Here's how the part is built. I have some questions about the finished solid (model axes, mm). A direction names the side the tool comes from. Round coordinates to 2 decimals unless told otherwise and drop trailing zeros. Loops run counter-clockwise (first coordinate to the right, second up) from the corner with the lowest first, then second, coordinate; pieces in that order, holes last. Notation, with made-up numbers: (71, 69) - (116, 69) arc R27 cw to (116, 89) - close; hole circle Ø1 at (88.25, 80.25). An arc over 180 degrees is marked (long way). Return JSON: item names as keys, results as strings. Group by question number.
```python
from build123d import *

# Parameters (mm, degrees)
BASE_PLATE_DEPTH               = 56
HUB_BOSS_PROFILE_R             = 25
HUB_BOSS_PROFILE_R_2           = 12.5
HUB_BOSS_27_DEPTH              = 33
HUB_BORE_PROFILE_R             = 12.5
HUB_BORE_DEPTH                 = 186.162091153
FLANGE_START                   = 5
FLANGE_PLATE_PROFILE_R         = 6
FLANGE_PLATE_DEPTH             = 5
BASE_MOUNTING_HOLE_1_PROFILE_R = 8
BASE_MOUNTING_HOLE_1_DEPTH     = 209.137574695
BASE_MOUNTING_HOLE_2_PROFILE_R = 8
BASE_MOUNTING_HOLE_2_DEPTH     = 209.137574695
HUB_TO_BASE_FILLET_R5_R        = 5
FLANGE_FILLET_R5_R             = 5


with BuildPart() as part:
    # Base Plate Profile → Base Plate (new body)
    with BuildSketch(Plane.XY):
        Polygon((0, 0), (75, 0), (165, 0), (165, 16), (0, 16), align=None)
    extrude(amount=BASE_PLATE_DEPTH)

    # Hub Boss Profile → Hub Boss Ø27 (add, symmetric)
    with BuildSketch(Plane.XY.offset(25)):
        with Locations((82.5, 27)):
            Circle(HUB_BOSS_PROFILE_R)
        with Locations((82.5, 27)):
            Circle(HUB_BOSS_PROFILE_R_2, mode=Mode.SUBTRACT)
    extrude(amount=HUB_BOSS_27_DEPTH, both=True)

    # Hub Bore Profile → Hub Bore (cut, through all)
    with BuildSketch(Plane.XY.offset(58)):
        with Locations((82.5, 27)):
            Circle(HUB_BORE_PROFILE_R)
    extrude(amount=-HUB_BORE_DEPTH, mode=Mode.SUBTRACT)

    # Flange Plate Profile → Flange Plate (add)
    # profile 1 of 2: a face of its own
    with BuildSketch(Plane.XY.offset(51).offset(FLANGE_START)):
        with BuildLine():
            ThreePointArc((82.5, 87), (71.893398282, 91.393398282), (67.5, 102))
            Line((67.5, 102), (67.5, 47))
            ThreePointArc((67.5, 47), (82.5, 52), (97.5, 47))
            Line((97.5, 47), (97.5, 85.094750193))
            ThreePointArc((97.5, 85.094750193), (90.060257549, 86.521781776), (82.5, 87))
        make_face()
    # profile 2 of 2: a face of its own
    with BuildSketch(Plane.XY.offset(51).offset(FLANGE_START)):
        with BuildLine():
            ThreePointArc((142.5, 27), (124.926406871, 69.426406871), (82.5, 87))
            ThreePointArc((82.5, 87), (67.5, 102), (82.5, 117))
            ThreePointArc((82.5, 117), (146.139610307, 90.639610307), (172.5, 27))
            ThreePointArc((172.5, 27), (157.5, 12), (142.5, 27))
        make_face()
        with Locations((120, 91.951905284)):
            Circle(FLANGE_PLATE_PROFILE_R, mode=Mode.SUBTRACT)
        with Locations((147.451905284, 64.5)):
            Circle(FLANGE_PLATE_PROFILE_R, mode=Mode.SUBTRACT)
        with Locations((157.5, 27)):
            Circle(FLANGE_PLATE_PROFILE_R, mode=Mode.SUBTRACT)
        with Locations((82.5, 102)):
            Circle(FLANGE_PLATE_PROFILE_R, mode=Mode.SUBTRACT)
    extrude(amount=-FLANGE_PLATE_DEPTH)

    # Base Mounting Hole 1 Profile → Base Mounting Hole 1 (cut, through all)
    with BuildSketch(Plane(origin=(0, 16, 0), x_dir=(1, 0, 0), z_dir=(0, 1, 0))):
        with Locations(Location((25, -25, 0), (0, 0, 270))):
            Circle(BASE_MOUNTING_HOLE_1_PROFILE_R)
    extrude(amount=-BASE_MOUNTING_HOLE_1_DEPTH, mode=Mode.SUBTRACT)

    # Base Mounting Hole 2 Profile → Base Mounting Hole 2 (cut, through all)
    with BuildSketch(Plane(origin=(0, 16, 0), x_dir=(1, 0, 0), z_dir=(0, 1, 0))):
        with Locations(Location((140, -25, 0), (0, 0, 270))):
            Circle(BASE_MOUNTING_HOLE_2_PROFILE_R)
    extrude(amount=-BASE_MOUNTING_HOLE_2_DEPTH, mode=Mode.SUBTRACT)

    # Hub to Base Fillet R5
    hub_to_base_fillet_r5_edges = [part.edges().sort_by_distance(p)[0] for p in [
        (60.050055679, 16, 28),
    ]]
    fillet(hub_to_base_fillet_r5_edges, radius=HUB_TO_BASE_FILLET_R5_R)

    # Flange Fillet R5
    flange_fillet_r5_edges = [part.edges().sort_by_distance(p)[0] for p in [
        (104.949944321, 16, 28),
        (147.301960973, 16, 53.5),
    ]]
    fillet(flange_fillet_r5_edges, radius=FLANGE_FILLET_R5_R)


solid = part.part
```
Q1. Imagine slicing it at D-D, the plane y = 64.5. List the corners of the cut face in (x, z) for me.
Q2. Imagine slicing it at A-A, the plane x = 25. List the corners of the cut face in (y, z) for me.
Q3. Imagine slicing it at C-C, the plane z = 25. List the corners of the cut face in (x, y) for me, and give its area (3 significant figures).
Q4. For faces 4 (the cylindrical face through (71.78, 112.49, 53.54)), 5 (the flat face through (97.5, 66, 54)), which set-ups out of +Z, -Z, +X, -X, +Y, -Y let a thin tool reach every point of the face, with its end or its side?
Q5. If we mould it in two halves opening along Y, with no side actions, what happens to faces 1 (the cylindrical face through (142.68, 24.69, 53.54)), 2 (the flat face through (81, 1, 0)), 3 (the flat face through (33, 16, 28))? For each: +Y half, -Y half, draft (parallel to the pull), parting line (faces both ways), or undercut.
Q6. Will these pins go through, and if not, where does the flat tip stop? pin 1 Ø12 at (y, z) = (15.5, 28) entering from +X; pin 2 Ø1.5 at (y, z) = (66.5, 54.5) entering from +X; pin 3 Ø19 at (x, y) = (157.5, 27) entering from +Z.
Q7. Please list where these lines run through material, in increasing order: line 1 (X direction, y = 7, z = 25); line 2 (Y direction, x = 120, z = 54); line 3 (Y direction, x = 19, z = 51).
Q8. Imagine slicing it at B-B, the plane y = 42. List the corners of the cut face in (x, z) for me, and give its area (3 significant figures).
Output values:
{
 "1": {"outline": "(67.5, 51) - (97.5, 51) - (97.5, 56) - (67.5, 56) - close; (129.34, 51) - (141.45, 51) - (141.45, 56) - (129.34, 56) - close; (153.45, 51) - (164.32, 51) - (164.32, 56) - (153.45, 56) - close"},
 "2": {"outline": "(0, 0) - (16, 0) - (16, 17) - (0, 17) - close; (0, 33) - (16, 33) - (16, 56) - (0, 56) - close"},
 "3": {"outline": "(0, 0) - (17, 0) - (17, 16) - (0, 16) - close; (33, 0) - (132, 0) - (132, 16) - (111.89, 16) arc R5 cw to (106.99, 22) arc R25 ccw (long way) to (58.01, 22) arc R5 cw to (53.11, 16) - (33, 16) - close; (148, 0) - (165, 0) - (165, 16) - (148, 16) - close; hole circle Ø25 at (82.5, 27)", "area": "3,170 mm^2"},
 "4": {"face 4": "+Z, -Z, -X, +Y", "face 5": "+Z, -Z"},
 "5": {"face 1": "undercut", "face 2": "draft", "face 3": "+Y half"},
 "6": {"pin 1": "stops at x = 165", "pin 2": "stops at x = 163.73", "pin 3": "stops at z = 56"},
 "7": {"line 1": "x = 0 to 17, 33 to 132, 148 to 165", "line 2": "y = 0 to 16, 73.84 to 85.95, 97.95 to 108.82", "line 3": "y = 0 to 16"},
 "8": {"outline": "(62.5, -8) - (102.5, -8) - (102.5, 58) - (62.5, 58) - close; (140.59, 51) - (171.24, 51) - (171.24, 56) - (140.59, 56) - close", "area": "2,790 mm^2"}
}
